from build123d import *

# Parameters (mm, degrees)
SKETCH_1_W          = 47
SKETCH_1_H          = 185
EXTRUDE_1_DEPTH     = 6
CHAMFER_1_SIZE      = 10
CUT_EXTRUDE_2_REACH = 193.254


with BuildPart() as part:
    # 草图1 → 凸台-拉伸1 (new, symmetric)
    with BuildSketch(Plane.XY):
        with Locations((23.5, 92.5)):
            Rectangle(SKETCH_1_W, SKETCH_1_H)
    extrude(amount=EXTRUDE_1_DEPTH, both=True)

    # 倒角1
    chamfer_1_edges = [part.edges().sort_by_distance(p)[0] for p in [
        (47, 185, 0),
    ]]
    chamfer(chamfer_1_edges, length=CHAMFER_1_SIZE)

    # 草图3 → 切除-拉伸2 (cut, up to next)
    with BuildSketch(Plane(origin=(0, 0, -6), x_dir=(-1, 0, 0), z_dir=(0, 0, -1)), mode=Mode.PRIVATE) as cut_extrude_2_sk1:
        with BuildLine():
            Line((-47, 81.5), (-41, 81.5))
            ThreePointArc((-41, 81.5), (-34.5, 75), (-41, 68.5))
            Line((-41, 68.5), (-47, 68.5))
            Line((-47, 68.5), (-47, 81.5))
        make_face()
    cut_extrude_2_tool1 = extrude(cut_extrude_2_sk1.sketch, amount=-CUT_EXTRUDE_2_REACH, mode=Mode.PRIVATE) & part.part
    add(cut_extrude_2_tool1.solids().sort_by_distance((41.352691, 75, -6))[0], mode=Mode.SUBTRACT)


solid = part.part
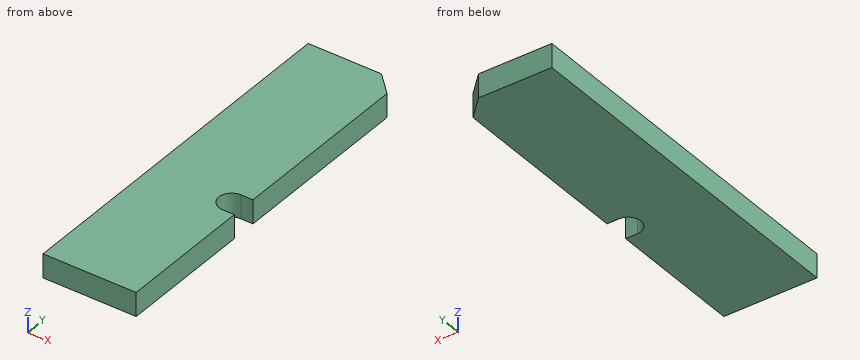
Geometry: final body of the model. Coordinates: model frame, mm. Give positions to 0.01 mm unless a question says otherwise; leave off trailing zeros. Loops run counter-clockwise (first coordinate to the right, second up) from the corner with the lowest first, then second, coordinate; pieces in that order, holes last. Notation, with made-up numbers: (60.25, 20) -> (87.25, 20) arc R29 ccw to (87.25, 54) -> close; hole circle Ø6 at (-39.5, 78). An arc over 180 degrees is marked (long way). Put each result on its own line as item: value.
1. Pin query (flat end, axial travel): P1, Ø1.8, axis at x = 43.5, z = 1.5, coming from the +Y side. Return the tip coordinate at first contact, or that it passes through.
Taken from the geometry:
P1: stops at y = 179.4
2. Cut plane A-A (z = -3.5). Return the cut outline in (x, y).
Taken from the geometry:
outline: (0, 0) -> (47, 0) -> (47, 68.5) -> (41, 68.5) arc R6.5 cw to (41, 81.5) -> (47, 81.5) -> (47, 175) -> (37, 185) -> (0, 185) -> close
3. Cut plane B-B (y = 75). Return the cut outline in (x, z), plus the area to 3 significant figures.
Taken from the geometry:
outline: (0, -6) -> (34.5, -6) -> (34.5, 6) -> (0, 6) -> close
area: 414 mm2
4. Ray query, line 1 along Y through (x, z) = (41.5, 0.5); line 2 along Y through (x, z) = (41, -5). Return the intervals inside material, ascending. Write a range as [from, to].
Taken from the geometry:
line 1: y = [0, 68.5], [81.5, 180.5]
line 2: y = [0, 68.5], [81.5, 181]
